Read the model definition and answer for the solid it produces. Units are mm, in the model's axes. A direction names the side the tool comes from. Coordinates: 2 decimals unless noted, no trailing zeros. Loops run counter-clockwise (first coordinate to the right, second up) from the corner with the lowest first, then second, coordinate; pieces in that order, holes last. Notation, with made-up numbers: (70, -37) -> (80, -37) arc R11 cw to (80, -26) -> close; hole circle Ø10 at (64, 47.5). An arc over 180 degrees is marked (long way). Answer as a JSON object with one key per item and string values. Group by question number.
1) Determine the mould class of faces 1 (the face through (0, -1, 1)), 2 (the face through (150, 0, 0)), 3 (the face through (126.506, 0.286, -0.385)) for opening direction X: released by +X, released by -X, zero draft, split by the parting line, or undercut.
2) Section D-D, the plane x = 34 is taken. Give the vertices of the cut face in (y, z), plus the area to 3 significant figures.
3) Which of the six approach directions +Z, -Z, +X, -X, +Y, -Y give full straight-line access (tool end or side, diameter ignored) to faces 4 (the face through (4.55, 46.37, -10.3)), 5 (the face through (45.5, -22, 17))?
4) Section A-A, the plane y = 0 is taken. Give the vertices of the cut face in (x, z), plus the area to 3 significant figures.
5) Consider probe 1 along X at (y, z) = (0, 3.5); probe 2 along X at (y, z) = (-7.5, 37); probe 3 along Y at (x, z) = (133, 13). Determine where each line is inside the solid, lowest interval first. Write a range as [from, to].
6) Flat-ended cylindrical pins translate along their axes: P1, Ø2, axis at x = 30.5, y = 7, coming from the +Z side; P2, Ø3, axis at y = -35.5, z = 19.5, coming from the +X side; P3, Ø3, axis at x = 61.5, z = -11, coming from the -Y side. Find the tip coordinate at first contact, or state that the pin passes through.
7) Section C-C, the plane x = 133 is taken. Give the vertices of the cut face in (y, z), plus the area to 3 significant figures.
8) Section B-B, the plane z = 0 is taken. Give the vertices of the cut face in (x, y), plus the area to 3 significant figures.
from build123d import *

# Parameters (mm, degrees)
FILLET1_R               = 1
CHAMFER1_SIZE           = 1
CUT_EXTRUDE1_DEPTH      = 165.354799139
CUT_EXTRUDE1_DEPTH_BACK = 165.354799139
SKETCH2_R               = 6.5


with BuildPart() as part:
    # Sketch1 → Revolve1 (revolve)
    with BuildSketch(Plane.XY, mode=Mode.PRIVATE) as revolve1_sk:
        Polygon((0, 0), (0, 47.5), (8, 47.5), (9.5, 46.633974596), (9.5, 30), (45.5, 30), (45.5, 27.5), (150, 27.5), (150, 0), align=None)
    revolve(revolve1_sk.sketch.rotate(Axis((0, 0, 0), (1, 0, 0)), 90), axis=Axis((0, 0, 0), (1, 0, 0)))

    # Fillet1
    fillet1_edges = [part.edges().sort_by_distance(p)[0] for p in [
        (9.5, 0, -30),
    ]]
    fillet(fillet1_edges, radius=FILLET1_R)

    # Chamfer1
    chamfer1_edges = [part.edges().sort_by_distance(p)[0] for p in [
        (150, 0, -27.5),
        (45.5, 0, -30),
        (0, 0, -47.5),
    ]]
    chamfer(chamfer1_edges, length=CHAMFER1_SIZE)

    # Sketch2 → Cut-Extrude1 (cut, two sides: drawn at the far end of the back side and taken through both)
    with BuildSketch(Plane.XY.offset(-CUT_EXTRUDE1_DEPTH_BACK)):
        with Locations((133, 0)):
            Circle(SKETCH2_R)
    extrude(amount=CUT_EXTRUDE1_DEPTH + CUT_EXTRUDE1_DEPTH_BACK, mode=Mode.SUBTRACT)


solid = part.part
Determined:
{
 "1": {"face 1": "released by -X", "face 2": "released by +X", "face 3": "undercut"},
 "2": {"outline": "circle Ø60 at (0, 0)", "area": "2,830 mm²"},
 "3": {"face 4": "+X, -X", "face 5": "+X"},
 "4": {"outline": "(0, -46.5) -> (1, -47.5) -> (8, -47.5) -> (9.5, -46.63) -> (9.5, -31) arc R1 cw to (10.5, -30) -> (44.5, -30) -> (45.5, -29) -> (45.5, -27.5) -> (126.5, -27.5) -> (126.5, 27.5) -> (45.5, 27.5) -> (45.5, 29) -> (44.5, 30) -> (10.5, 30) arc R1 cw to (9.5, 31) -> (9.5, 46.63) -> (8, 47.5) -> (1, 47.5) -> (0, 46.5) -> close; (139.5, -27.5) -> (149, -27.5) -> (150, -26.5) -> (150, 26.5) -> (149, 27.5) -> (139.5, 27.5) -> close", "area": "8,090 mm²"},
 "5": {"probe 1": "[0, 126.5], [139.5, 150]", "probe 2": "[0, 9.5]", "probe 3": "[-24.23, -6.5], [6.5, 24.23]"},
 "6": {"P1": "z = 29.39", "P2": "x = 9.5", "P3": "y = -25.81"},
 "7": {"outline": "(-6.5, -26.72) -> (-6.5, 26.72) arc R27.5 ccw to start; (6.5, -26.72) arc R27.5 ccw to (6.5, 26.72) -> close", "area": "1,670 mm²"},
 "8": {"outline": "(0, -46.5) -> (1, -47.5) -> (8, -47.5) -> (9.5, -46.63) -> (9.5, -31) arc R1 cw to (10.5, -30) -> (44.5, -30) -> (45.5, -29) -> (45.5, -27.5) -> (149, -27.5) -> (150, -26.5) -> (150, 26.5) -> (149, 27.5) -> (45.5, 27.5) -> (45.5, 29) -> (44.5, 30) -> (10.5, 30) arc R1 cw to (9.5, 31) -> (9.5, 46.63) -> (8, 47.5) -> (1, 47.5) -> (0, 46.5) -> close; hole circle Ø13 at (133, 0)", "area": "8,670 mm²"}
}
